```python
from build123d import *

# Parameters (mm, degrees)
EXTRUDE_1_DEPTH          = 80
SKETCH_4_W               = 520
SKETCH_4_H               = 50
EXTRUDE_2_DEPTH          = 2125
EXTRUDE_3_DEPTH          = 80
CUT_EXTRUDE_3_DEPTH      = 2638.351891576
CUT_EXTRUDE_3_DEPTH_BACK = 2638.351891576
SKETCH_2_R               = 210
EXTRUDE_4_DEPTH          = 100
SKETCH_7_R               = 20
CUT_EXTRUDE_5_DEPTH      = 20
CUT_EXTRUDE_6_DEPTH      = 100
CUT_REVOLVE_1_ANGLE      = 90


with BuildPart() as part:
    # 草图1 → 凸台-拉伸1 (new body)
    with BuildSketch(Plane.XY):
        Polygon((0, 0), (0, -1000), (2125, -1000), (2125, -630), (1600, 0), align=None)
    extrude(amount=EXTRUDE_1_DEPTH)

    # 草图4 → 凸台-拉伸2 (add)
    with BuildSketch(Plane(origin=(0, 0, 0), x_dir=(0, 0, -1), z_dir=(1, 0, 0))):
        with Locations((-340, -975)):
            Rectangle(SKETCH_4_W, SKETCH_4_H)
    extrude_2 = extrude(amount=EXTRUDE_2_DEPTH)

    # 镜向4: 凸台-拉伸2 across plane
    add(extrude_2.mirror(Plane.XY.offset(600)))

    # 草图5 → 凸台-拉伸3 (add)
    with BuildSketch(Plane.XY.offset(1120)):
        Polygon((0, -1000), (0, 0), (1600, 0), (2125, -630), (2125, -1000), align=None)
    extrude(amount=EXTRUDE_3_DEPTH)

    # 草图2 → 切除-拉伸3 (cut, two sides: drawn at the far end of the back side and taken through both)
    with BuildSketch(Plane.XY.offset(-CUT_EXTRUDE_3_DEPTH_BACK)):
        with Locations(Location((410, -420, 0), (0, 0, 180))):
            Circle(SKETCH_2_R)
    extrude(amount=CUT_EXTRUDE_3_DEPTH + CUT_EXTRUDE_3_DEPTH_BACK, mode=Mode.SUBTRACT)

    # 草图6 → 凸台-拉伸4 (add)
    with BuildSketch(Plane.XY):
        Polygon((800.5, -500), (2125, -815), (2125, -785), (800.5, -470), align=None)
    extrude_4 = extrude(amount=EXTRUDE_4_DEPTH)

    # 镜向5: 凸台-拉伸4 across plane
    add(extrude_4.mirror(Plane.XY.offset(600)))

    # 草图7 → 切除-拉伸5 (cut)
    with BuildSketch(Plane.XY):
        with Locations((170, -420)):
            Circle(SKETCH_7_R)
        with Locations((289.999999999, -627.846096908)):
            Circle(SKETCH_7_R)
        with Locations((530.000000001, -627.846096908)):
            Circle(SKETCH_7_R)
        with Locations((650, -420)):
            Circle(SKETCH_7_R)
        with Locations((289.999999999, -212.153903092)):
            Circle(SKETCH_7_R)
        with Locations((530.000000001, -212.153903092)):
            Circle(SKETCH_7_R)
    cut_extrude_5 = extrude(amount=CUT_EXTRUDE_5_DEPTH, mode=Mode.SUBTRACT)

    # 镜向6: 切除-拉伸5 across plane
    add(cut_extrude_5.mirror(Plane.XY.offset(600)), mode=Mode.SUBTRACT)

    # 草图8 → 切除-拉伸6 (cut)
    with BuildSketch(Plane(origin=(2125, 0, 0), x_dir=(0, 0, -1), z_dir=(1, 0, 0))):
        with BuildLine():
            Line((-1200, -860), (-1180, -860))
            ThreePointArc((-1180, -860), (-1140, -820), (-1180, -780))
            Line((-1180, -780), (-1200, -780))
            Line((-1200, -780), (-1200, -860))
        make_face()
    cut_extrude_6 = extrude(amount=-CUT_EXTRUDE_6_DEPTH, mode=Mode.SUBTRACT)

    # 草图9 → 切除-旋转1 (revolve, cut)
    with BuildSketch(Plane.XY.offset(1200)):
        with BuildLine():
            Line((2025, -760), (2025, -880))
            ThreePointArc((2025, -880), (1965, -820), (2025, -760))
        make_face()
    cut_revolve_1 = revolve(axis=Axis((2025, -760, 1200), (0, -1, 0)), revolution_arc=CUT_REVOLVE_1_ANGLE, mode=Mode.SUBTRACT)

    # 镜向7: 切除-拉伸6, 切除-旋转1 across plane
    add(cut_extrude_6.mirror(Plane.XY.offset(600)), mode=Mode.SUBTRACT)
    add(cut_revolve_1.mirror(Plane.XY.offset(600)), mode=Mode.SUBTRACT)


solid = part.part
```
The listing builds one solid part. Answer for the finished solid, in the listing's coordinates (mm). A direction names the side the tool comes from. Give positions to 0.01 mm unless a question says otherwise; leave off trailing zeros. Loops run counter-clockwise (first coordinate to the right, second up) from the corner with the lowest first, then second, coordinate; pieces in that order, holes last. Notation, with made-up numbers: M -15.75,39.5 L 39.25,39.5 A25 ccw 39.25,71.5 Z; hole C -13.5,4.25 d11. An arc over 180 degrees is marked long. One line per item, written item: value.
1. Find the intervals of material crossed by probe 1 along Z at (x, y) = (295.5, -690); probe 2 along Y at (x, z) = (410, 1183.5); probe 3 along Y at (x, z) = (650, 7.5), in increasing order.
Found:
probe 1: 0 to 80, 1120 to 1200
probe 2: -1000 to -630, -210 to 0
probe 3: -1000 to -440, -400 to 0
2. Section D-D on x = 1038 is taken. Determine the outline of the cut face in (y, z).
Found:
outline: M -1000,0 L 0,0 L 0,80 L -526.48,80 L -526.48,100 L -556.48,100 L -556.48,80 L -950,80 L -950,1120 L -556.48,1120 L -556.48,1100 L -526.48,1100 L -526.48,1120 L 0,1120 L 0,1200 L -1000,1200 Z
3. Each of these flat-tipped pins is pushed along its axis until it touches: P1, Ø20, axis at x = 532, y = -634, coming from the -Z side; P2, Ø6, axis at y = -490.5, z = 1109.5, coming from the -X side; P3, Ø4, axis at x = 848.5, z = 499, coming from the +Y side. Where does it stop, or does it pass through?
Found:
P1: z = 20
P2: x = 800.5
P3: y = -950
4. Section B-B on y = -693.5 is taken. Determine the outline of the cut face in (x, z), plus the area to 3 significant figures.
Found:
outline: M 0,0 L 2125,0 L 2125,80 L 1740.26,80 L 1740.26,100 L 1614.12,100 L 1614.12,80 L 0,80 Z; M 0,1120 L 1614.12,1120 L 1614.12,1100 L 1740.26,1100 L 1740.26,1120 L 2125,1120 L 2125,1200 L 0,1200 Z
area: 345,000 mm^2
5. For a pull along X with two mould halves and no side action, classify faces 4 (the face through (1472, -629.7, 1110.1)), 5 (the face through (313.098, -233.694, 1159.44)), 6 (the face through (2075.7, -820.88, 59.99)) as pulls with the +X half, pulls with the -X half, needs draft (parallel to the pull), parting line crosses it, or undercut.
Found:
face 4: pulls with the +X half
face 5: undercut
face 6: needs draft
6. Section A-A on x = 410 is taken. Determine the outline of the cut face in (y, z).
Found:
outline: M -1000,0 L -630,0 L -630,80 L -950,80 L -950,1120 L -630,1120 L -630,1200 L -1000,1200 Z; M -210,0 L 0,0 L 0,80 L -210,80 Z; M -210,1120 L 0,1120 L 0,1200 L -210,1200 Z
7. For faces 1 (the face through (515.26, -614.33, 9.86)), 2 (the face through (290, -212, 1180)), 3 (the face through (2075.7, -820.88, 1140.01)), determine the directions among +Z, -Z, +X, -X, +Y, -Y from which every point of the face is accessible in a straight line to the end or side of a thin tool.
Found:
face 1: -Z
face 2: +Z
face 3: +Z, +X
8. Section C-C on y = -534.5 is taken. Determine the outline of the cut face in (x, z), plus the area to 3 significant figures.
Found:
outline: M 0,0 L 233.96,0 L 233.96,80 L 0,80 Z; M 0,1120 L 233.96,1120 L 233.96,1200 L 0,1200 Z; M 586.04,0 L 2045.42,0 L 2045.42,80 L 1071.71,80 L 1071.71,100 L 945.56,100 L 945.56,80 L 586.04,80 Z; M 586.04,1120 L 945.56,1120 L 945.56,1100 L 1071.71,1100 L 1071.71,1120 L 2045.42,1120 L 2045.42,1200 L 586.04,1200 Z
area: 276,000 mm^2
